Check sheet for the modelled part. Datum: model origin and axes. Units: mm. A direction names the side the tool comes from. Round coordinates to 2 decimals unless told otherwise and drop trailing zeros. Loops run counter-clockwise (first coordinate to the right, second up) from the corner with the lowest first, then second, coordinate; pieces in that order, holes last. Notation, with made-up numbers: (22.5, -9) - (66.5, -9) arc R15 ccw to (66.5, 4) - close; hole circle Ø7 at (-8.75, 65). An arc over 180 degrees is marked (long way). Put each result on its own line as item: value. Start each with the question number.
Item 1: Material ranges on line 1 along Y through (x, z) = (-18.5, 295.5); line 2 along Y through (x, z) = (41, 585), recorded low to high.
Item 2: Draft check along X on faces 3 (the flat face through (-50, 1, 597)), 4 (the flat face through (1, 50, 597)), 5 (the flat face through (-45.5, 1, 597)). Enter one of: pulls with the +X half, pulls with the -X half, needs draft (parallel to the pull), parting line crosses it, or undercut.
Item 3: Section check A-A, the plane z = 300.5. Record the cut outline in (x, y), and give its area (3 significant figures).
Item 4: Gauge pin test, flat ends, axial feed: pin 1 Ø9 at (x, z) = (0, 1191) entering from -Y; pin 2 Ø2 at (x, z) = (-47, 30.5) entering from -Y; pin 3 Ø2 at (x, z) = (-48, 16) entering from +Y. Record the tip position at first contact, or that the pin passes through.
Item 5: Tool access check on faces 1 (the flat face through (-1, -45.5, 597)), 2 (the flat face through (0, -46, 0)). Record the directions out of +Z, -Z, +X, -X, +Y, -Y that give a thin tool (end or side, any length) a straight path to the whole face; none if there is none.
from build123d import *

# Parameters (mm, degrees)
BOSS_EXTRUDE1_DEPTH = 1211
CUT_EXTRUDE1_REACH  = 1218.15
SKETCH_1_R          = 7.5
CUT_EXTRUDE2_REACH  = 1218.15
SKETCH2_R           = 7.5
CUT_EXTRUDE3_REACH  = 1218.15
SKETCH3_R           = 7.5
SKETCH4_W           = 45
SKETCH4_H           = 9
CUT_EXTRUDE4_DEPTH  = 1217.150072976


with BuildPart() as part:
    # Sketch1 → Boss-Extrude1 (new body)
    with BuildSketch(Plane.XY):
        with BuildLine():
            Line((-40, -50), (40, -50))
            ThreePointArc((40, -50), (47.071067812, -47.071067812), (50, -40))
            Line((50, -40), (50, 40))
            ThreePointArc((50, 40), (47.071067812, 47.071067812), (40, 50))
            Line((40, 50), (-40, 50))
            ThreePointArc((-40, 50), (-47.071067812, 47.071067812), (-50, 40))
            Line((-50, 40), (-50, -40))
            ThreePointArc((-50, -40), (-47.071067812, -47.071067812), (-40, -50))
        make_face()
        with BuildLine():
            Line((-40, -45.5), (40, -45.5))
            ThreePointArc((40, -45.5), (43.889087297, -43.889087297), (45.5, -40))
            Line((45.5, -40), (45.5, 40))
            ThreePointArc((45.5, 40), (43.889087297, 43.889087297), (40, 45.5))
            Line((40, 45.5), (-40, 45.5))
            ThreePointArc((-40, 45.5), (-43.889087297, 43.889087297), (-45.5, 40))
            Line((-45.5, 40), (-45.5, -40))
            ThreePointArc((-45.5, -40), (-43.889087297, -43.889087297), (-40, -45.5))
        make_face(mode=Mode.SUBTRACT)
    extrude(amount=BOSS_EXTRUDE1_DEPTH)

    # 草图1 → Cut-Extrude1 (cut, up to next)
    with BuildSketch(Plane(origin=(50, 0, 0), x_dir=(0, 0, -1), z_dir=(1, 0, 0)), mode=Mode.PRIVATE) as cut_extrude1_sk1:
        with Locations((-1171, -15)):
            Circle(SKETCH_1_R)
    cut_extrude1_tool1 = extrude(cut_extrude1_sk1.sketch, amount=-CUT_EXTRUDE1_REACH, mode=Mode.PRIVATE) & part.part
    # 草图1 → Cut-Extrude1 (cut, up to next)
    with BuildSketch(Plane(origin=(50, 0, 0), x_dir=(0, 0, -1), z_dir=(1, 0, 0)), mode=Mode.PRIVATE) as cut_extrude1_sk2:
        with Locations((-1121, -15)):
            Circle(SKETCH_1_R)
    cut_extrude1_tool2 = extrude(cut_extrude1_sk2.sketch, amount=-CUT_EXTRUDE1_REACH, mode=Mode.PRIVATE) & part.part
    add(cut_extrude1_tool1.solids().sort_by_distance((50, -15, 1171))[0], mode=Mode.SUBTRACT)
    add(cut_extrude1_tool2.solids().sort_by_distance((50, -15, 1121))[0], mode=Mode.SUBTRACT)

    # Sketch2 → Cut-Extrude2 (cut, up to next)
    with BuildSketch(Plane.XZ.offset(50), mode=Mode.PRIVATE) as cut_extrude2_sk1:
        with Locations(Location((0, 1191, 0), (0, 0, 270))):
            Circle(SKETCH2_R)
    cut_extrude2_tool1 = extrude(cut_extrude2_sk1.sketch, amount=-CUT_EXTRUDE2_REACH, mode=Mode.PRIVATE) & part.part
    # Sketch2 → Cut-Extrude2 (cut, up to next)
    with BuildSketch(Plane.XZ.offset(50), mode=Mode.PRIVATE) as cut_extrude2_sk2:
        with Locations(Location((0, 1121, 0), (0, 0, 270))):
            Circle(SKETCH2_R)
    cut_extrude2_tool2 = extrude(cut_extrude2_sk2.sketch, amount=-CUT_EXTRUDE2_REACH, mode=Mode.PRIVATE) & part.part
    # Sketch2 → Cut-Extrude2 (cut, up to next)
    with BuildSketch(Plane.XZ.offset(50), mode=Mode.PRIVATE) as cut_extrude2_sk3:
        with Locations(Location((0, 20, 0), (0, 0, 270))):
            Circle(SKETCH2_R)
    cut_extrude2_tool3 = extrude(cut_extrude2_sk3.sketch, amount=-CUT_EXTRUDE2_REACH, mode=Mode.PRIVATE) & part.part
    add(cut_extrude2_tool1.solids().sort_by_distance((0, -50, 1191))[0], mode=Mode.SUBTRACT)
    add(cut_extrude2_tool2.solids().sort_by_distance((0, -50, 1121))[0], mode=Mode.SUBTRACT)
    add(cut_extrude2_tool3.solids().sort_by_distance((0, -50, 20))[0], mode=Mode.SUBTRACT)

    # Sketch3 → Cut-Extrude3 (cut, up to next)
    with BuildSketch(Plane(origin=(0, 50, 0), x_dir=(1, 0, 0), z_dir=(0, 1, 0)), mode=Mode.PRIVATE) as cut_extrude3_sk1:
        with Locations(Location((-15, -1171, 0), (0, 0, 270))):
            Circle(SKETCH3_R)
    cut_extrude3_tool1 = extrude(cut_extrude3_sk1.sketch, amount=-CUT_EXTRUDE3_REACH, mode=Mode.PRIVATE) & part.part
    # Sketch3 → Cut-Extrude3 (cut, up to next)
    with BuildSketch(Plane(origin=(0, 50, 0), x_dir=(1, 0, 0), z_dir=(0, 1, 0)), mode=Mode.PRIVATE) as cut_extrude3_sk2:
        with Locations(Location((-15, -1121, 0), (0, 0, 270))):
            Circle(SKETCH3_R)
    cut_extrude3_tool2 = extrude(cut_extrude3_sk2.sketch, amount=-CUT_EXTRUDE3_REACH, mode=Mode.PRIVATE) & part.part
    add(cut_extrude3_tool1.solids().sort_by_distance((-15, 50, 1171))[0], mode=Mode.SUBTRACT)
    add(cut_extrude3_tool2.solids().sort_by_distance((-15, 50, 1121))[0], mode=Mode.SUBTRACT)

    # Sketch4 → Cut-Extrude4 (cut, through all)
    with BuildSketch(Plane(origin=(50, 0, 0), x_dir=(0, 0, -1), z_dir=(1, 0, 0))):
        with Locations((-22.5, 0)):
            Rectangle(SKETCH4_W, SKETCH4_H)
    extrude(amount=-CUT_EXTRUDE4_DEPTH, mode=Mode.SUBTRACT)


solid = part.part
Check result:
1. line 1: -50 to -45.5, 45.5 to 50
1. line 2: -49.95 to -45.41, 45.41 to 49.95
2. face 3: pulls with the -X half
2. face 4: needs draft
2. face 5: undercut
3. outline: (-50, -40) arc R10 ccw to (-40, -50) - (40, -50) arc R10 ccw to (50, -40) - (50, 40) arc R10 ccw to (40, 50) - (-40, 50) arc R10 ccw to (-50, 40) - close; hole (-45.5, -40) arc R5.5 ccw to (-40, -45.5) - (40, -45.5) arc R5.5 ccw to (45.5, -40) - (45.5, 40) arc R5.5 ccw to (40, 45.5) - (-40, 45.5) arc R5.5 ccw to (-45.5, 40) - close
3. area: 1,660 mm²
4. pin 1: y = 45.5
4. pin 2: y = -48
4. pin 3: y = 47.14
5. face 1: +Z, -Z
5. face 2: -Z, +X, -X, +Y, -Y
